Part model, mm, in its own coordinate system. A direction names the side the tool comes from. Round coordinates to 2 decimals unless told otherwise and drop trailing zeros. Loops run counter-clockwise (first coordinate to the right, second up) from the corner with the lowest first, then second, coordinate; pieces in that order, holes last. Notation, with made-up numbers: M -36.5,88 L 4.5,88 A3 ccw 4.5,93 Z; hole C 79,27.5 d6. An arc over 180 degrees is marked long. Put each result on its own line as item: value. Start each with the question number.
```python
from build123d import *

# Parameters (mm, degrees)
SKETCH1_R           = 6.5
BOSS_EXTRUDE1_DEPTH = 8


with BuildPart() as part:
    # Sketch1 → Boss-Extrude1 (new body)
    with BuildSketch(Plane.XY):
        with BuildLine():
            Line((0, 0), (170, 0))
            ThreePointArc((170, 0), (189.359816102, -9.182366786), (194.498117616, -29.98419836))
            Line((194.498117616, -29.98419836), (177.204672165, -114.98419836))
            ThreePointArc((177.204672165, -114.98419836), (168.524187763, -129.359816102), (152.706554549, -135))
            Line((152.706554549, -135), (17.293445451, -135))
            ThreePointArc((17.293445451, -135), (1.475812237, -129.359816102), (-7.204672165, -114.98419836))
            Line((-7.204672165, -114.98419836), (-24.498117616, -29.98419836))
            ThreePointArc((-24.498117616, -29.98419836), (-19.359816102, -9.182366786), (0, 0))
        make_face()
        with Locations((0, -25)):
            Circle(SKETCH1_R, mode=Mode.SUBTRACT)
        with Locations((170, -25)):
            Circle(SKETCH1_R, mode=Mode.SUBTRACT)
        with BuildLine():
            Line((14.81381342, -103.878677575), (42.81381342, -93.878677575))
            ThreePointArc((42.81381342, -93.878677575), (51.121322425, -97.81381342), (47.18618658, -106.121322425))
            Line((47.18618658, -106.121322425), (19.18618658, -116.121322425))
            ThreePointArc((19.18618658, -116.121322425), (10.878677575, -112.18618658), (14.81381342, -103.878677575))
        make_face(mode=Mode.SUBTRACT)
        with BuildLine():
            Line((127.18618658, -93.878677575), (155.18618658, -103.878677575))
            ThreePointArc((155.18618658, -103.878677575), (159.121322425, -112.18618658), (150.81381342, -116.121322425))
            Line((150.81381342, -116.121322425), (122.81381342, -106.121322425))
            ThreePointArc((122.81381342, -106.121322425), (118.878677575, -97.81381342), (127.18618658, -93.878677575))
        make_face(mode=Mode.SUBTRACT)
    extrude(amount=BOSS_EXTRUDE1_DEPTH)


solid = part.part
```
1. Wall check: L1, parallel to X at y = -30.5, z = 7.75; L2, parallel to Y at x = 143, z = 6.75; L3, parallel to Y at x = 0, z = 2. Give the ranges that are in metal, low to high.
2. Cut at D-D, the plane y = -100. Give the cut face in (x, z).
3. Cut at A-A, the plane y = -25. Give the cut face in (x, z), and give its area (3 significant figures).
4. Which spindle directions (+Z, -Z, +X, -X, +Y, -Y) get a long thin tool onto all of the face, cutting with end or side? Do faces 1 (the flat face through (185.972, -71.889, 3.944)), 2 (the flat face through (28.62, -98.95, 3.94)). Say none if no direction does.
5. Mould opens along X. For faces 3 (the cylindrical face through (168.709, -129.207, 3.944)), 4 (the flat face through (87, -67, 0)), 5 (the cylindrical face through (159.17, -112.05, 3.94)) say: released by +X, released by -X, zero draft, split by the parting line, or undercut.
6. Cut at C-C, the plane z = 4.75. Give the cut face in (x, y), and give its area (3 significant figures).
7. Cut at B-B, the plane x = 125. Give the cut face in (y, z), and give its area (3 significant figures).
8. Drop flat-ended pins along their axis: pin 1 (2 mm diameter, centred on y = -49, z = 4.5, fed in from +X); pin 2 (4 mm diameter, centred on y = -53, z = 3, fed in from -X). Give the stop position or say it passes through.
Results list:
1. L1: x = -24.39 to -3.46, 3.46 to 166.54, 173.46 to 194.39
1. L2: y = -135 to -113.33, -99.53 to 0
1. L3: y = -128.05 to -31.5, -18.5 to 0
2. outline: M -10.25,0 L 25.67,0 L 25.67,8 L -10.25,8 Z; M 51.5,0 L 118.5,0 L 118.5,8 L 51.5,8 Z; M 144.33,0 L 180.25,0 L 180.25,8 L 144.33,8 Z
3. outline: M -25,0 L -6.5,0 L -6.5,8 L -25,8 Z; M 6.5,0 L 163.5,0 L 163.5,8 L 6.5,8 Z; M 176.5,0 L 195,0 L 195,8 L 176.5,8 Z
3. area: 1,550 mm^2
4. face 1: +Z, -Z, +X, -Y
4. face 2: +Z, -Z
5. face 3: released by +X
5. face 4: zero draft
5. face 5: undercut
6. outline: M -24.5,-29.98 L -7.2,-114.98 A25 ccw 17.29,-135 L 152.71,-135 A25 ccw 177.2,-114.98 L 194.5,-29.98 A25 ccw 170,0 L 0,0 A25 ccw Z; hole C 0,-25 d13; hole M 14.81,-103.88 A6.5 ccw 19.19,-116.12 L 47.19,-106.12 A6.5 ccw 42.81,-93.88 Z; hole M 122.81,-106.12 L 150.81,-116.12 A6.5 ccw 155.19,-103.88 L 127.19,-93.88 A6.5 ccw Z; hole C 170,-25 d13
6. area: 25,600 mm^2
7. outline: M -135,0 L -106.9,0 L -106.9,8 L -135,8 Z; M -93.5,0 L 0,0 L 0,8 L -93.5,8 Z
7. area: 973 mm^2
8. pin 1: stops at x = 190.83
8. pin 2: stops at x = -20.22
